Here's how the part is built. I have some questions about the finished solid (model axes, mm). Face numbers are marked on the shaded views. A direction names the side the tool comes from. Coordinates: 2 decimals unless noted, no trailing zeros. Order: outer loops, then holes, each group sorted by start corner. A loop starts at its lowest first (then second) coordinate and runs counter-clockwise, first axis right, second up. Notation, with made-up numbers: (67.5, 74.25) -> (99.5, 74.25) arc R27 cw to (99.5, 101.25) -> close; hole circle Ø6 at (-0.75, 14.5). An arc over 180 degrees is marked (long way). One line per item, written item: value. Start each with the question number.
```python
from build123d import *

# Parameters (mm, degrees)
BOSS_EXTRUDE1_DEPTH       = 18
CHAMFER1_SIZE             = 2
M8X1_0_TAPPED_HOLE1_D     = 7
M8X1_0_TAPPED_HOLE1_DEPTH = 13
M8X1_0_TAPPED_HOLE1_TIP   = 2.103012167
HOLE2_D                   = 9
SKETCH15_R                = 32.5
CUT_EXTRUDE3_DEPTH        = 2.5
CUT_EXTRUDE4_START        = -2.5
SKETCH16_R                = 32.5
CUT_EXTRUDE4_DEPTH        = 2.5
HOLE3_D                   = 4


with BuildPart() as part:
    # Sketch1 → Boss-Extrude1 (new body)
    with BuildSketch(Plane.XY):
        with BuildLine():
            Line((-50, 24), (-33, 24))
            Line((-33, 24), (-33, 47))
            Line((-33, 47), (33, 47))
            Line((33, 47), (33, 24))
            Line((33, 24), (50, 24))
            Line((50, 24), (50, 0))
            Line((50, 0), (30, 0))
            ThreePointArc((30, 0), (0, 30), (-30, 0))
            Line((-30, 0), (-50, 0))
            Line((-50, 0), (-50, 24))
        make_face()
    extrude(amount=BOSS_EXTRUDE1_DEPTH)

    # Chamfer1
    chamfer1_edges = [part.edges().sort_by_distance(p)[0] for p in [
        (-50, 24, 9),
        (-33, 47, 9),
        (33, 47, 9),
        (50, 24, 9),
    ]]
    chamfer(chamfer1_edges, length=CHAMFER1_SIZE)

    # M8x1.0 Tapped Hole1
    with Locations(Plane(origin=(0, 47, 0), x_dir=(1, 0, 0), z_dir=(0, 1, 0))):
        with Locations((0, -9)):
            Hole(M8X1_0_TAPPED_HOLE1_D / 2, depth=M8X1_0_TAPPED_HOLE1_DEPTH)
            with Locations((0, 0, -(M8X1_0_TAPPED_HOLE1_DEPTH + M8X1_0_TAPPED_HOLE1_TIP / 2))):  # 118° drill point
                Cone(0, M8X1_0_TAPPED_HOLE1_D / 2, M8X1_0_TAPPED_HOLE1_TIP, mode=Mode.SUBTRACT)

    # Hole2 (through all)
    with Locations(Plane(origin=(0, 24, 0), x_dir=(1, 0, 0), z_dir=(0, 1, 0))):
        with Locations((-41, -9), (41, -9)):
            Hole(HOLE2_D / 2)

    # Sketch15 → Cut-Extrude3 (cut)
    with BuildSketch(Plane(origin=(0, 0, 0), x_dir=(-1, 0, 0), z_dir=(0, 0, -1))):
        Circle(SKETCH15_R)
    extrude(amount=-CUT_EXTRUDE3_DEPTH, mode=Mode.SUBTRACT)

    # Sketch16 → Cut-Extrude4 (cut)
    with BuildSketch(Plane.XY.offset(18).offset(CUT_EXTRUDE4_START)):
        Circle(SKETCH16_R)
    extrude(amount=CUT_EXTRUDE4_DEPTH, mode=Mode.SUBTRACT)

    # Hole3 (through all)
    with Locations(Plane(origin=(0, 47, 0), x_dir=(1, 0, 0), z_dir=(0, 1, 0))):
        with Locations((0, -9)):
            Hole(HOLE3_D / 2)


solid = part.part
```
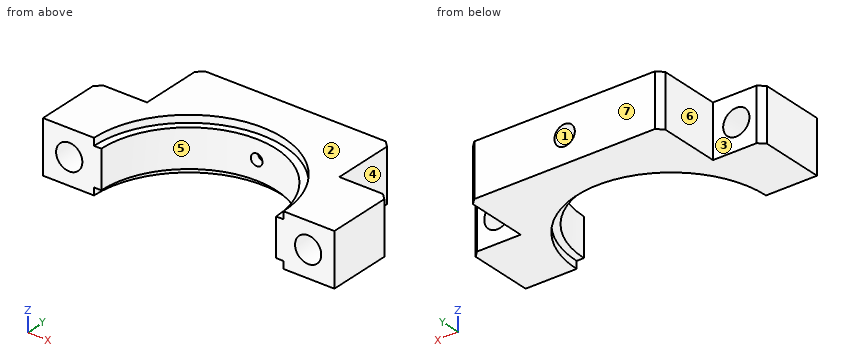
Q1. Imagine slicing it at C-C (x = 41). Write out the boundary of the cut face in (y, z), plus the area to 3 significant figures.
Q2. For the marked faces 1, 2, 3 and 4, which set-ups out of +Z, -Z, +X, -X, +Y, -Y let a thin tool reach every point of the face, with its end or its side?
Q3. For P1, Ø5.5, axis at y = 29.5, z = 11, coming from the +X side; P2, Ø7.5, axis at x = 37.5, z = 9, coming from the +Y side; P3, Ø10, axis at y = 26, z = 7, coming from the -X side; P4, Ø5, axis at x = 0, z = 9, coming from the -Y side, each with a flat end and sliding along its axis, tell me the tip position at first contact or that it passes through.
Q4. Imagine slicing it at A-A (y = 7). Write out the boundary of the cut face in (x, z), plus the area to 3 significant figures.
Q5. If we mould it in two halves opening along X, with no side actions, what happens to the marked faces 5, 6 and 7? For each: +X half, -X half, draft (parallel to the pull), parting line (faces both ways), or undercut.
Q6. I need wall thicknesses on line 1 (X direction, y = 37.5, z = 9); line 2 (Z direction, x = -41, y = 9); line 3 (Z direction, x = 0, y = 31.2). Which ranges of each line are inside material? Lowest first, please.
Q7. Imagine slicing it at B-B (z = 9). Count the separate pieces of the cut face and the enclosed holes in it, plus the area to 3 significant figures.
Q8. Imagine slicing it at D-D (y = 28.5). Write out the boundary of the cut face in (x, z), plus the area to 3 significant figures.
Completed:
1. outline: (0, 0) -> (24, 0) -> (24, 4.5) -> (0, 4.5) -> close; (0, 13.5) -> (24, 13.5) -> (24, 18) -> (0, 18) -> close
1. area: 216 mm2
2. face 1: +Y
2. face 2: +Z, +X, -X, +Y, -Y
2. face 3: +Z, -Z, -X, +Y
2. face 4: +Z, -Z, +X, +Y
3. P1: stops at x = 33
3. P2: stops at y = 24
3. P3: stops at x = -50
3. P4: stops at y = 29.9
4. outline: (-50, 0) -> (-31.74, 0) -> (-31.74, 2.5) -> (-29.17, 2.5) -> (-29.17, 15.5) -> (-31.74, 15.5) -> (-31.74, 18) -> (-50, 18) -> close; (29.17, 2.5) -> (31.74, 2.5) -> (31.74, 0) -> (50, 0) -> (50, 18) -> (31.74, 18) -> (31.74, 15.5) -> (29.17, 15.5) -> close; hole circle Ø9 at (-41, 9); hole circle Ø9 at (41, 9)
4. area: 597 mm2
5. face 5: undercut
5. face 6: -X half
5. face 7: draft
6. line 1: x = -33 to -3.5, 3.5 to 33
6. line 2: z = 0 to 4.5, 13.5 to 18
6. line 3: z = 2.5 to 7, 11 to 15.5
7. separate pieces: 4
7. enclosed holes: 0
7. area: 1,960 mm2
8. outline: (-33, 0) -> (-15.62, 0) -> (-15.62, 2.5) -> (-9.37, 2.5) -> (-9.37, 15.5) -> (-15.62, 15.5) -> (-15.62, 18) -> (-33, 18) -> close; (9.37, 2.5) -> (15.62, 2.5) -> (15.62, 0) -> (33, 0) -> (33, 18) -> (15.62, 18) -> (15.62, 15.5) -> (9.37, 15.5) -> close
8. area: 788 mm2
